Here's the drawing with two shaded views (mm, measured from the low corner). I have some questions. A direction names the side the tool comes from. Coordinates: 2 decimals unless noted, no trailing zeros. Order: outer loops, then holes, each group sorted by start corner. A loop starts at its lowest first (then second) coordinate and runs counter-clockwise, first axis right, second up. Notation, with made-up numbers: (-12.5, 34.5) - (12.5, 34.5) arc R20 cw to (12.5, 62.5) - close; hole circle Ø11 at (88.25, 58). An arc over 180 degrees is marked (long way). Answer as CSV lines item,"result". Start each with the question number.
1. I want a section at A-A, the plane y = 29. List the corners of the cut face in (x, z) for me.
2. For pin 1 (2 mm diameter, centred on x = 51.5, y = 44.5, fed in from +Z); pin 2 (1 mm diameter, centred on y = 38.5, z = 10, fed in from -X); pin 3 (1.5 mm diameter, centred on x = 14, z = 10, fed in from +Y), each with a flat end and sliding along its axis, tell me the tip position at first contact or that it passes through.
3. I need wall thicknesses on probe 1 along X at (y, z) = (28.5, 2); probe 2 along Y at (x, z) = (20, 7.5); probe 3 along X at (y, z) = (31.5, 10). Which ranges of each line are inside material? Lowest first, please.
4. I want a section at C-C, the plane z = 1.5. List the corners of the cut face in (x, y) for me.
5. Thinking about a two-plate mould opening in X: for the marked faces 1, 2 and 3, which applies, released by +X, released by -X, zero draft, split by the parting line, or undercut?
6. I want a section at B-B, the plane x = 29. List the corners of the cut face in (y, z) for me, and give its area (3 significant figures).
7. I want a section at D-D, the plane x = 38. List the corners of the cut face in (y, z) for me, and give its area (3 significant figures).
8. For the marked faces 4 and 5, which set-ups out of +Z, -Z, +X, -X, +Y, -Y let a thin tool reach every point of the face, with its end or its side?
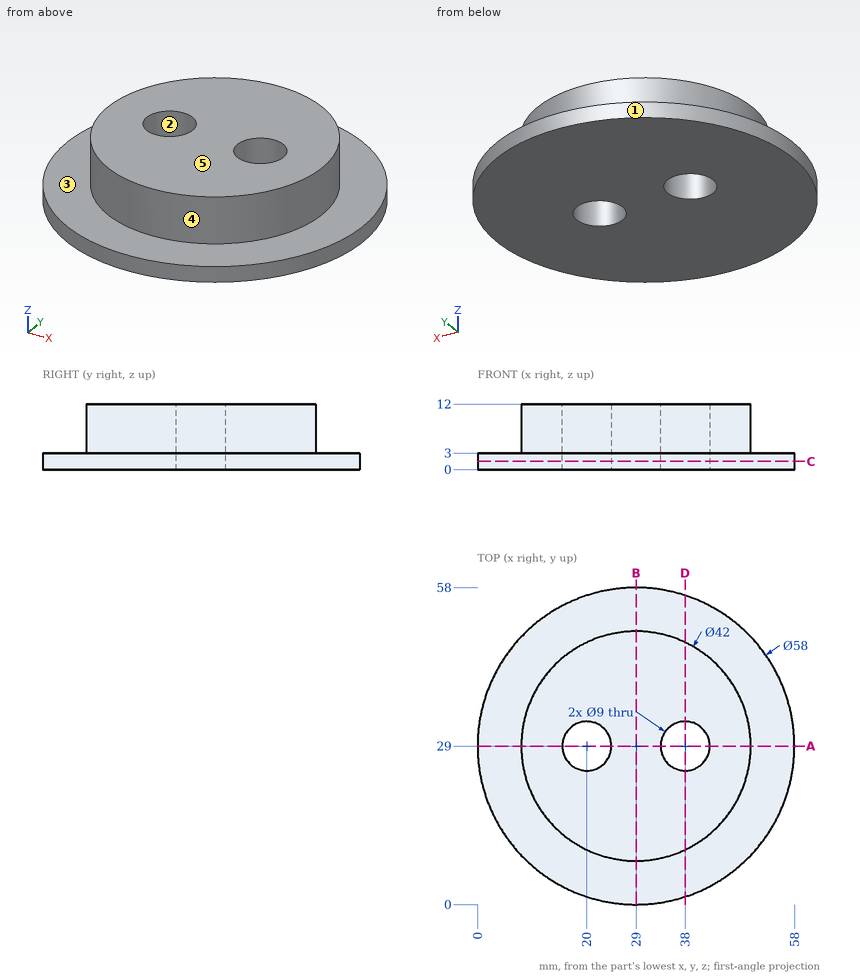
Solved:
1,outline,"(0, 0) - (15.5, 0) - (15.5, 12) - (8, 12) - (8, 3) - (0, 3) - close; (24.5, 0) - (33.5, 0) - (33.5, 12) - (24.5, 12) - close; (42.5, 0) - (58, 0) - (58, 3) - (50, 3) - (50, 12) - (42.5, 12) - close"
2,pin 1,"stops at z = 3"
2,pin 2,"stops at x = 10.03"
2,pin 3,"stops at y = 44.43"
3,probe 1,"x = 0 to 15.53, 24.47 to 33.53, 42.47 to 58"
3,probe 2,"y = 10.03 to 24.5, 33.5 to 47.97"
3,probe 3,"x = 8.15 to 16.26, 23.74 to 34.26, 41.74 to 49.85"
4,outline,"circle Ø58 at (29, 29); hole circle Ø9 at (20, 29); hole circle Ø9 at (38, 29)"
5,face 1,"split by the parting line"
5,face 2,"undercut"
5,face 3,"zero draft"
6,outline,"(0, 0) - (58, 0) - (58, 3) - (50, 3) - (50, 12) - (8, 12) - (8, 3) - (0, 3) - close"
6,area,"552 mm2"
7,outline,"(1.43, 0) - (24.5, 0) - (24.5, 12) - (10.03, 12) - (10.03, 3) - (1.43, 3) - close; (33.5, 0) - (56.57, 0) - (56.57, 3) - (47.97, 3) - (47.97, 12) - (33.5, 12) - close"
7,area,"399 mm2"
8,face 4,"+Z"
8,face 5,"+Z, +X, -X, +Y, -Y"
